from build123d import *


with BuildPart() as part:
    # 草图1 → 旋转1 (revolve)
    with BuildSketch(Plane.XY, mode=Mode.PRIVATE) as revolve_1_sk:
        Polygon((-4, 13.7), (-4, 11.75), (-3.6, 11.75), (-3.6, 8.75), (-4, 8.75), (-4, 6.3), (-3.7, 6), (3.7, 6), (4, 6.3), (4, 8.75), (3.6, 8.75), (3.6, 11.75), (4, 11.75), (4, 13.7), (3.7, 14), (-3.7, 14), align=None)
    revolve(revolve_1_sk.sketch.rotate(Axis((4, 0, 0), (-1, 0, 0)), 270), axis=Axis((4, 0, 0), (-1, 0, 0)))


solid = part.part
Source: CAD feature listing. Evaluate the final solid. Frame: model axes, mm. A direction names the side the tool comes from. Give positions to 0.01 mm unless a question says otherwise; leave off trailing zeros. Write each loop counter-clockwise with the first axis right and the second up, starting at its lowest first coordinate (ties: lowest second). Pieces come first, ordered by that corner, then holes. Notation, with made-up numbers: M -13.75,-11 L -8.75,-11 A6 ccw -8.75,-7 Z; hole C -19,42 d3. An arc over 180 degrees is marked long. Answer as a JSON object with one key per item and string values.
Q1. Mould query, pull axis Z, two halves, no side actions, for faces 1 (the face through (3.8, 7.9, -8.7)), 2 (the face through (4, -4, -6)), 3 (the face through (-3.803, -5.324, -6.944)), 4 (the face through (-0.05, -13.67, -3.03)). Classes: +Z half, -Z half, draft (parallel to the pull), parting line (faces both ways), or undercut.
Geometry check:
{"face 1": "undercut", "face 2": "draft", "face 3": "undercut", "face 4": "parting line"}
Q2. Contact query for flat-ended pins moving along their axis: P1, Ø2, axis at x = -0.5, y = -7, coming from the -Z side; P2, Ø4, axis at x = 2, y = 5, coming from the -Z side; P3, Ø4, axis at x = 2, z = 3, coming from the +Y side; P4, Ø7, axis at y = -0.5, z = 0, coming from the -X side. Output: stop coordinate, or through.
Geometry check:
{"P1": "stops at z = -12.65", "P2": "stops at z = -13.67", "P3": "stops at y = 13.96", "P4": "passes through"}
Q3. Ray query, line 1 along Y through (x, z) = (1.75, 0); line 2 along Y through (x, z) = (3.75, 0); line 3 along Z through (x, y) = (0, -2.75). Return the intervals inside material, ascending.
Geometry check:
{"line 1": "y = -14 to -6, 6 to 14", "line 2": "y = -13.95 to -11.75, -8.75 to -6.05, 6.05 to 8.75, 11.75 to 13.95", "line 3": "z = -13.73 to -5.33, 5.33 to 13.73"}
Q4. Cut plane C-C, the plane x = 3. Return the cut outline in (y, z), then the cut area to 3 significant figures.
Geometry check:
{"outline": "C 0,0 d28; hole C 0,0 d12", "area": "503 mm^2"}
Q5. Access query for faces 5 (the face through (3.797, -5.324, -6.944)), 6 (the face through (-3.6, 9, 0)), 7 (the face through (0.052, 1.802, 5.723)). Directions: +Z, -Z, +X, -X, +Y, -Y. A direction counts if a zero-diameter tool reaches every point of the face in a straight line with its end or side. Return the directions, or none.
Geometry check:
{"face 5": "+X", "face 6": "-X", "face 7": "+X, -X"}
